Part print with two shaded views. Sizes in mm from the minimum x, y, z corner. A direction names the side the tool comes from. Give positions to 0.01 mm unless a question says otherwise; leave off trailing zeros. Loops run counter-clockwise (first coordinate to the right, second up) from the corner with the lowest first, then second, coordinate; pieces in that order, holes last. Notation, with made-up numbers: (32, -7.5) -> (50, -7.5) arc R19 cw to (50, 1.5) -> close; hole circle Ø11 at (25.5, 86). An arc over 180 degrees is marked (long way). One line per question, with ' | ' between items. Start each with the question number.
(1) Flat gauge pins, fed straight in: pin 1 Ø9.5 at (x, y) = (15, 15) entering from +Z; pin 2 Ø1.5 at (x, y) = (40.5, 41.5) entering from -Z; pin 3 Ø4 at (y, z) = (73.5, 41) entering from +X; pin 4 Ø15 at (x, z) = (24, 22) entering from -Y. Where does each tip first touch, or does it go through?
(2) Drill centre lines: L1, parallel to Y at x = 55, z = 55.25; L2, parallel to Z at x = 24, y = 58; L3, parallel to X at y = 12, z = 53. Where is each one in solid material? Low to high. Write a range as from..to.
(3) Slice it at D-D, the plane z = 16. Write the cut outline in (x, y), then the cut area to 3 significant figures.
(4) Slice it at C-C, the plane y = 41.5. Write the cut outline in (x, z).
(5) Slice it at A-A, the plane x = 15. Write the cut outline in (y, z), then the cut area to 3 significant figures.
(6) Mould opens along Y. For the marked faces 3, 4 and 5 say: pulls with the +Y half, pulls with the -Y half, needs draft (parallel to the pull), parting line crosses it, or undercut.
(7) 3-axis set-ups, long thin cutter, end or side, ignore diameter. For the marked faces 1 and 2: which of +Z, -Z, +X, -X, +Y, -Y reach the whole face in a straight line?
(8) Slice it at B-B, the plane z = 56. Write the cut outline in (x, y).
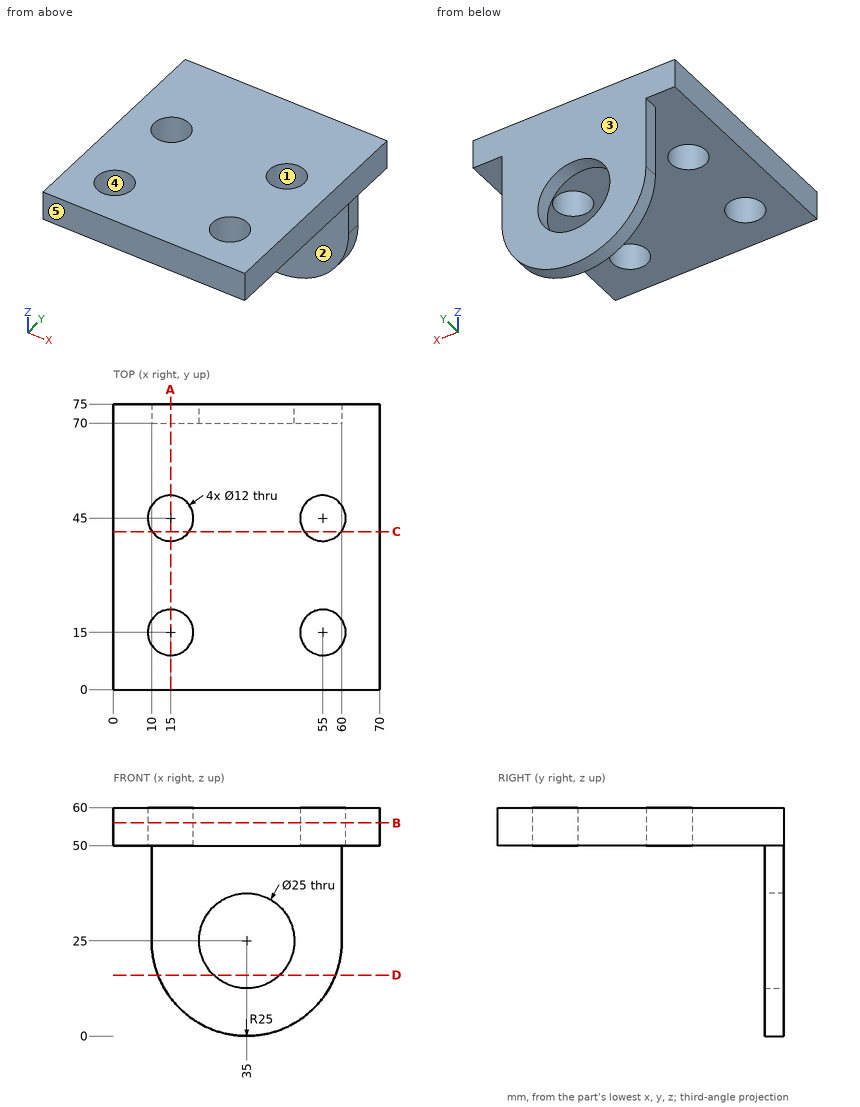
Final values:
1) pin 1: through | pin 2: z = 50 | pin 3: x = 60 | pin 4: y = 70
2) L1: 0..9, 21..39, 51..75 | L2: 50..60 | L3: 0..9.8, 20.2..49.8, 60.2..70
3) outline: (11.68, 70) -> (26.33, 70) -> (26.33, 75) -> (11.68, 75) -> close; (43.67, 70) -> (58.32, 70) -> (58.32, 75) -> (43.67, 75) -> close | area: 146 mm2
4) outline: (0, 50) -> (10.13, 50) -> (10.13, 60) -> (0, 60) -> close; (19.87, 50) -> (50.13, 50) -> (50.13, 60) -> (19.87, 60) -> close; (59.87, 50) -> (70, 50) -> (70, 60) -> (59.87, 60) -> close
5) outline: (0, 50) -> (9, 50) -> (9, 60) -> (0, 60) -> close; (21, 50) -> (39, 50) -> (39, 60) -> (21, 60) -> close; (51, 50) -> (70, 50) -> (70, 10) -> (75, 10) -> (75, 60) -> (51, 60) -> close | area: 710 mm2
6) face 3: pulls with the +Y half | face 4: undercut | face 5: pulls with the -Y half
7) face 1: +Z, -Z | face 2: -Z, +X, -X, -Y
8) outline: (0, 0) -> (70, 0) -> (70, 75) -> (0, 75) -> close; hole circle Ø12 at (15, 15); hole circle Ø12 at (15, 45); hole circle Ø12 at (55, 15); hole circle Ø12 at (55, 45)
